```python
from build123d import *

# Parameters (mm, degrees)
BASE_FLANGE_SKETCH_W     = 180
BASE_FLANGE_SKETCH_H     = 140
BASE_FLANGE_SKETCH_R     = 35
BASE_FLANGE_SKETCH_R_2   = 10
BASE_FLANGE_5MM_DEPTH    = 5
SIDE_GUSSET_SKETCH_R     = 25
SIDE_GUSSET_SKETCH_R_2   = 10
SIDE_GUSSET_SKETCH_W     = 5
SIDE_GUSSET_SKETCH_H     = 140
SIDE_GUSSET_A_DEPTH      = 5
SIDE_START               = -175
SKETCH2_5_R              = 25
SKETCH2_5_R_2            = 10
SKETCH2_5_W              = 5
SKETCH2_5_H              = 140
SIDE_GUSSET_B_DEPTH      = 5
BASE_FLANGE_FILLET_R10_R = 10
GUSSET_EDGE_FILLET_R10_R = 10
BACK_PLATE_SKETCH_W      = 5
BACK_PLATE_SKETCH_H      = 145
BACK_PLATE_DEPTH         = 15
MOTOR_MOUNT_PAD_SKETCH_R = 10
MOTOR_MOUNT_PAD_SKETCH_W = 5
MOTOR_MOUNT_PAD_SKETCH_H = 145
MOTOR_MOUNT_PAD_DEPTH    = 5
MOUNT_EDGE_FILLET_R10_R  = 10


with BuildPart() as part:
    # Base Flange Sketch → Base Flange 5mm (new body)
    with BuildSketch(Plane.XY):
        Rectangle(BASE_FLANGE_SKETCH_W, BASE_FLANGE_SKETCH_H)
        Circle(BASE_FLANGE_SKETCH_R, mode=Mode.SUBTRACT)
        with Locations((-45, 45)):
            Circle(BASE_FLANGE_SKETCH_R_2, mode=Mode.SUBTRACT)
        with Locations((45, 45)):
            Circle(BASE_FLANGE_SKETCH_R_2, mode=Mode.SUBTRACT)
        with Locations((-45, -45)):
            Circle(BASE_FLANGE_SKETCH_R_2, mode=Mode.SUBTRACT)
        with Locations((45, -45)):
            Circle(BASE_FLANGE_SKETCH_R_2, mode=Mode.SUBTRACT)
    extrude(amount=BASE_FLANGE_5MM_DEPTH)

    # Side Gusset Sketch → Side Gusset A (add)
    # profile 1 of 2: a face of its own
    with BuildSketch(Plane.ZY.offset(90)):
        Polygon((35, 70), (5, 70), (5, -70), (160, -70), (160, -50), (133.569366052, -24.626591409), (97.5, 10), (61.430633948, 44.626591409), align=None)
        with Locations((62.873408591, -26.069366052)):
            Circle(SIDE_GUSSET_SKETCH_R, mode=Mode.SUBTRACT)
        with Locations((119.718729488, -39.05433783)):
            Circle(SIDE_GUSSET_SKETCH_R_2, mode=Mode.SUBTRACT)
        with Locations((47.579997385, 30.198844989)):
            Circle(SIDE_GUSSET_SKETCH_R_2, mode=Mode.SUBTRACT)
    # profile 2 of 2: a face of its own
    with BuildSketch(Plane.ZY.offset(90)):
        with Locations((2.5, 0)):
            Rectangle(SIDE_GUSSET_SKETCH_W, SIDE_GUSSET_SKETCH_H)
    extrude(amount=-SIDE_GUSSET_A_DEPTH)

    # Sketch2_5 → Side Gusset B (add)
    # profile 1 of 2: a face of its own
    with BuildSketch(Plane.ZY.offset(90).offset(SIDE_START)):
        Polygon((35, 70), (5, 70), (5, -70), (160, -70), (160, -50), (133.569366052, -24.626591409), (97.5, 10), (61.430633948, 44.626591409), align=None)
        with Locations((62.873408591, -26.069366052)):
            Circle(SKETCH2_5_R, mode=Mode.SUBTRACT)
        with Locations((119.718729488, -39.05433783)):
            Circle(SKETCH2_5_R_2, mode=Mode.SUBTRACT)
        with Locations((47.579997385, 30.198844989)):
            Circle(SKETCH2_5_R_2, mode=Mode.SUBTRACT)
    # profile 2 of 2: a face of its own
    with BuildSketch(Plane.ZY.offset(90).offset(SIDE_START)):
        with Locations((2.5, 0)):
            Rectangle(SKETCH2_5_W, SKETCH2_5_H)
    extrude(amount=-SIDE_GUSSET_B_DEPTH)

    # Base Flange Fillet R10
    base_flange_fillet_r10_edges = [part.edges().sort_by_distance(p)[0] for p in [
        (-90, 0, 0),
        (90, 0, 0),
    ]]
    fillet(base_flange_fillet_r10_edges, radius=BASE_FLANGE_FILLET_R10_R)

    # Gusset Edge Fillet R10
    gusset_edge_fillet_r10_edges = [part.edges().sort_by_distance(p)[0] for p in [
        (-85, 0, 5),
        (85, 0, 5),
    ]]
    fillet(gusset_edge_fillet_r10_edges, radius=GUSSET_EDGE_FILLET_R10_R)

    # Back Plate Sketch → Back Plate (add)
    with BuildSketch(Plane.XZ.offset(70)):
        with Locations((-87.5, 87.5)):
            Rectangle(BACK_PLATE_SKETCH_W, BACK_PLATE_SKETCH_H)
        with Locations((87.5, 87.5)):
            Rectangle(BACK_PLATE_SKETCH_W, BACK_PLATE_SKETCH_H)
    extrude(amount=BACK_PLATE_DEPTH)

    # Motor Mount Pad Sketch → Motor Mount Pad (add)
    # profile 1 of 3: a face of its own
    with BuildSketch(Plane.XZ.offset(85)):
        with BuildLine():
            Line((-25.4, 160), (-85, 160))
            Line((-85, 160), (-85, 15))
            Line((-85, 15), (-25.4, 15))
            ThreePointArc((-25.4, 15), (-5.555268835, 30.543037168), (-15.891300301, 53.533596382))
            ThreePointArc((-15.891300301, 53.533596382), (-16.443437096, 53.797427747), (-16.991195266, 54.070233572))
            ThreePointArc((-16.991195266, 54.070233572), (-37.5, 87.5), (-16.991195266, 120.929766428))
            ThreePointArc((-16.991195266, 120.929766428), (-16.443437096, 121.202572253), (-15.891300301, 121.466403618))
            ThreePointArc((-15.891300301, 121.466403618), (-5.555268835, 144.456962832), (-25.4, 160))
        make_face()
        with Locations(Location((-25.4, 35.44, 0), (0, 0, 270))):
            Circle(MOTOR_MOUNT_PAD_SKETCH_R, mode=Mode.SUBTRACT)
        with Locations(Location((-25.4, 139.56, 0), (0, 0, 270))):
            Circle(MOTOR_MOUNT_PAD_SKETCH_R, mode=Mode.SUBTRACT)
    # profile 2 of 3: a face of its own
    with BuildSketch(Plane.XZ.offset(85)):
        with BuildLine():
            Line((90, 160), (25.4, 160))
            ThreePointArc((25.4, 160), (5.555268835, 144.456962832), (15.891300301, 121.466403618))
            ThreePointArc((15.891300301, 121.466403618), (16.443437096, 121.202572253), (16.991195266, 120.929766428))
            ThreePointArc((16.991195266, 120.929766428), (37.5, 87.5), (16.991195266, 54.070233572))
            ThreePointArc((16.991195266, 54.070233572), (16.443437096, 53.797427747), (15.891300301, 53.533596382))
            ThreePointArc((15.891300301, 53.533596382), (5.555268835, 30.543037168), (25.4, 15))
            Line((25.4, 15), (90, 15))
            Line((90, 15), (90, 160))
        make_face()
        with Locations(Location((25.4, 35.44, 0), (0, 0, 270))):
            Circle(MOTOR_MOUNT_PAD_SKETCH_R, mode=Mode.SUBTRACT)
        with Locations(Location((25.4, 139.56, 0), (0, 0, 270))):
            Circle(MOTOR_MOUNT_PAD_SKETCH_R, mode=Mode.SUBTRACT)
    # profile 3 of 3: a face of its own
    with BuildSketch(Plane.XZ.offset(85)):
        with Locations((-87.5, 87.5)):
            Rectangle(MOTOR_MOUNT_PAD_SKETCH_W, MOTOR_MOUNT_PAD_SKETCH_H)
    extrude(amount=-MOTOR_MOUNT_PAD_DEPTH)

    # Mount Edge Fillet R10
    mount_edge_fillet_r10_edges = [part.edges().sort_by_distance(p)[0] for p in [
        (85, -80, 87.5),
        (90, -85, 87.5),
        (-90, -85, 87.5),
        (-85, -80, 87.5),
    ]]
    fillet(mount_edge_fillet_r10_edges, radius=MOUNT_EDGE_FILLET_R10_R)


solid = part.part
```
Build history of the part. All positions in model axes, mm. A direction names the side the tool comes from. Round coordinates to 2 decimals unless told otherwise and drop trailing zeros. Loops run counter-clockwise (first coordinate to the right, second up) from the corner with the lowest first, then second, coordinate; pieces in that order, holes last.
Item 1: Saw through at A-A (x = 45). List the corners of the cut face in (y, z), then the cut area to 4 significant figures.
Item 2: Which spindle directions (+Z, -Z, +X, -X, +Y, -Y) get a long thin tool onto all of the face, cutting with end or side? Do faces 5 (the face through (47, -80, 89)), 6 (the face through (64, -81, 15)), 7 (the face through (5.65, -82.54, 144.83)). Say none if no direction does.
Item 3: Pin check, flat tips, straight feed: P1, Ø6, axis at x = -34, z = 114.5, coming from the +Y side; P2, Ø10, axis at x = -55.5, y = -49.5, coming from the +Z side. Stop position of each tip, or through.
Item 4: Saw through at D-D (y = 52.5). List the corners of the cut face in (x, z).
Item 5: Saw through at C-C (z = 117.5). List the corners of the cut face in (x, y).
Item 6: Saw through at B-B (x = 0). List the corners of the cut face in (y, z), then the cut area to 3 significant figures.
Item 7: Drill centre lines: line 1 along Y through (x, z) = (-45, 3.55); line 2 along X through (y, z) = (45.5, 18); line 3 along Z through (x, y) = (33, -42.5). Where is each one in solid material? Low to high.
Item 8: Two-plate mould, pull along Z, no slides. Class faces 1 (the face through (28.4, -82.54, 130.02)), 2 (the face through (-67, -81, 160)), 3 (the face through (-28, -21, 2)), 4 (the face through (87.465, -36.051, 129.257)): released by +Z, released by -Z, zero draft, split by the parting line, or undercut.
Worked answers:
1. outline: (-85, 15) - (-80, 15) - (-80, 160) - (-85, 160) - close; (-70, 0) - (-55, 0) - (-55, 5) - (-70, 5) - close; (-35, 0) - (35, 0) - (35, 5) - (-35, 5) - close; (55, 0) - (70, 0) - (70, 5) - (55, 5) - close
1. area: 1,225 mm2
2. face 5: +Z, -Z, +Y
2. face 6: -Z, +X, -X, -Y
2. face 7: +Y, -Y
3. P1: stops at y = -80
3. P2: stops at z = 5
4. outline: (-90, 10) arc R10 ccw to (-80, 0) - (-51.61, 0) - (-51.61, 5) - (-75, 5) arc R10 cw to (-85, 15) - (-85, 53.23) - (-90, 53.23) - close; (-38.39, 0) - (38.39, 0) - (38.39, 5) - (-38.39, 5) - close; (51.61, 0) - (80, 0) arc R10 ccw to (90, 10) - (90, 53.23) - (85, 53.23) - (85, 15) arc R10 cw to (75, 5) - (51.61, 5) - close
5. outline: (-90, -75) arc R10 ccw to (-80, -85) - (-22.5, -85) - (-22.5, -80) - (-75, -80) arc R10 cw to (-85, -70) - (-85, -48.81) - (-90, -48.81) - close; (-90, -29.3) - (-85, -29.3) - (-85, -9.2) - (-90, -9.2) - close; (22.5, -85) - (80, -85) arc R10 ccw to (90, -75) - (90, -48.81) - (85, -48.81) - (85, -70) arc R10 cw to (75, -80) - (22.5, -80) - close; (85, -29.3) - (90, -29.3) - (90, -9.2) - (85, -9.2) - close
6. outline: (-70, 0) - (-35, 0) - (-35, 5) - (-70, 5) - close; (35, 0) - (70, 0) - (70, 5) - (35, 5) - close
6. area: 350 mm2
7. line 1: y = -70 to -55, -35 to 35, 55 to 70
7. line 2: x = -90 to -85, 85 to 90
7. line 3: z = 0 to 5
8. face 1: undercut
8. face 2: released by +Z
8. face 3: zero draft
8. face 4: undercut
